Design review of the part built by this model. Coordinates are the model's own, in mm. Face numbers are marked on the shaded views. A direction names the side the tool comes from. Coordinates: 2 decimals unless noted, no trailing zeros. Order: outer loops, then holes, each group sorted by start corner. A loop starts at its lowest first (then second) coordinate and runs counter-clockwise, first axis right, second up. Notation, with made-up numbers: M -1.75,-8.5 L 16.25,-8.5 A3 cw 16.25,-3.5 Z; hole C 8.25,-1.5 d8. An arc over 180 degrees is marked long. Answer as a JSON object with one key per item and string values.
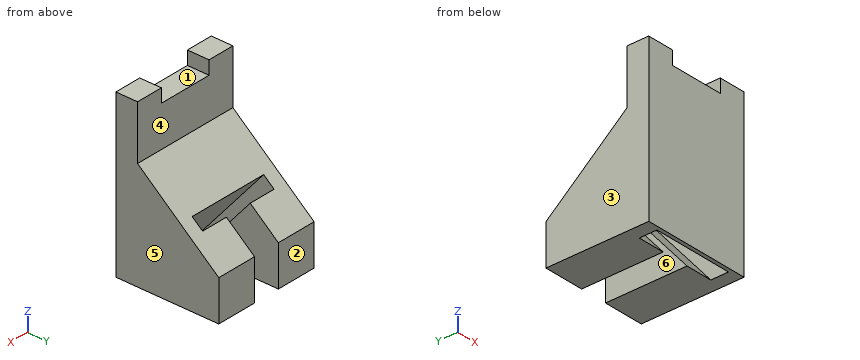
from build123d import *

# Parameters (mm, degrees)
BASE_PLATE_SKETCH_W                   = 40
BASE_PLATE_SKETCH_H                   = 60
BASE_PLATE_60X40X8_DEPTH              = 8
BASE_NOTCH_SKETCH_W                   = 20
BASE_NOTCH_SKETCH_H                   = 5
BASE_NOTCH_20X5_DEPTH                 = 20
UPRIGHT_BLOCK_SKETCH_W                = 40
UPRIGHT_BLOCK_SKETCH_H                = 30
UPRIGHT_BLOCK_40X30X40_DEPTH          = 40
SLOPED_FACE_CUT_DEPTH                 = 40
TOP_SLOT_CUT_DEPTH                    = 39
ANGLED_SLOT_THROUGH_SLOPED_FACE_REACH = 54.383
ANGLED_SLOT_SKETCH_W                  = 10
ANGLED_SLOT_SKETCH_H                  = 15


with BuildPart() as part:
    # Base Plate Sketch → Base Plate 60x40x8 (new body)
    with BuildSketch(Plane(origin=(0, 0, 0), x_dir=(1, 0, 0), z_dir=(0, 1, 0))):
        Rectangle(BASE_PLATE_SKETCH_W, BASE_PLATE_SKETCH_H)
    extrude(amount=BASE_PLATE_60X40X8_DEPTH)

    # Base Notch Sketch → Base Notch 20x5 (cut)
    with BuildSketch(Plane(origin=(0, 8, 0), x_dir=(1, 0, 0), z_dir=(0, 1, 0))):
        with Locations((0, -27.5)):
            Rectangle(BASE_NOTCH_SKETCH_W, BASE_NOTCH_SKETCH_H)
    extrude(amount=-BASE_NOTCH_20X5_DEPTH, mode=Mode.SUBTRACT)

    # Upright Block Sketch → Upright Block 40x30x40 (add)
    with BuildSketch(Plane(origin=(20, 0, 0), x_dir=(0, 0, -1), z_dir=(1, 0, 0))):
        with Locations((10, 23)):
            Rectangle(UPRIGHT_BLOCK_SKETCH_W, UPRIGHT_BLOCK_SKETCH_H)
    extrude(amount=-UPRIGHT_BLOCK_40X30X40_DEPTH)

    # Slope Cut Sketch → Sloped Face Cut (cut)
    with BuildSketch(Plane(origin=(20, 0, 0), x_dir=(0, 0, -1), z_dir=(1, 0, 0))):
        Polygon((15, 38), (-10, 38), (-10, 8), align=None)
    extrude(amount=-SLOPED_FACE_CUT_DEPTH, mode=Mode.SUBTRACT)

    # Top Slot Sketch → Top Slot Cut (cut)
    with BuildSketch(Plane(origin=(0, 8.196721311, 9.836065574), x_dir=(1, 0, 0), z_dir=(0, 0.6401843996644799, 0.768221279597376))):
        Polygon((-5, 25.272676797), (-15, 25.272676797), (-15, 20.272676797), (15, 20.272676797), (15, 25.272676797), (5, 25.272676797), (5, 38.79517462), (-5, 38.79517462), align=None)
    extrude(amount=-TOP_SLOT_CUT_DEPTH, mode=Mode.SUBTRACT)

    # Angled Slot Sketch → Angled Slot Through Sloped Face (cut, up to next)
    with BuildSketch(Plane(origin=(0, 38, 0), x_dir=(1, 0, 0), z_dir=(0, 1, 0)), mode=Mode.PRIVATE) as angled_slot_through_sloped_face_sk1:
        with Locations((0, 22.5)):
            Rectangle(ANGLED_SLOT_SKETCH_W, ANGLED_SLOT_SKETCH_H)
    angled_slot_through_sloped_face_tool1 = extrude(angled_slot_through_sloped_face_sk1.sketch, amount=-ANGLED_SLOT_THROUGH_SLOPED_FACE_REACH, mode=Mode.PRIVATE) & part.part
    add(angled_slot_through_sloped_face_tool1.solids().sort_by_distance((0, 38, -22.5))[0], mode=Mode.SUBTRACT)


solid = part.part
1) Insertion check: pin 1 Ø6 at (x, z) = (-7, 6.5) entering from +Y; pin 2 Ø2.5 at (x, y) = (3, 3) entering from +Z; pin 3 Ø16 at (x, z) = (6, 20.5) entering from +Y. Each pin has a flat end and moves straight along its axis. Give the tip position at first contact, or say it passes through.
Taken from the geometry:
{"pin 1": "stops at y = 15.8", "pin 2": "stops at z = 25", "pin 3": "stops at y = 8"}
2) To check wall thickness, follow L1, parallel to X at y = 29.5, z = -25; L2, parallel to X at y = 10, z = -22; L3, parallel to Y at x = -15.5, z = 18. State the ranges of each line that lie inside material, in increasing order.
Taken from the geometry:
{"L1": "x = -20 to -5, 5 to 20", "L2": "x = -20 to -15, 15 to 20", "L3": "y = 0 to 8"}
3) Mouldability with a two-part tool opening along X and no side actions: class the marked faces 1, 2 and 3 as released by +X, released by -X, zero draft, split by the parting line, or undercut.
Taken from the geometry:
{"face 1": "undercut", "face 2": "zero draft", "face 3": "released by -X"}
4) Add section A-A (x = 13). State the section outline as (y, z) points.
Taken from the geometry:
{"outline": "M 0,-30 L 1.39,-30 L 23.77,-3.14 L 8,10 L 8,30 L 0,30 Z; M 7.9,-30 L 38,-30 L 38,-15 L 27.61,-6.34 Z"}
5) Add section C-C (z = -9.5). State the section outline as (x, y) points.
Taken from the geometry:
{"outline": "M -20,0 L 20,0 L 20,31.4 L 5,31.4 L 5,24.98 L 15,24.98 L 15,18.47 L -15,18.47 L -15,24.98 L -5,24.98 L -5,31.4 L -20,31.4 Z"}
6) Tool access review of the marked faces 4, 5 and 6: name each direction out of +Z, -Z, +X, -X, +Y, -Y from which nothing blocks a thin tool from reaching the whole face with its end or side.
Taken from the geometry:
{"face 4": "+Z, +X, -X, +Y", "face 5": "+Z, -Z, +X, +Y, -Y", "face 6": "-Z, +Y"}
7) Add section D-D (x = 1.5). State the section outline as (y, z) points, and give its area (3 significant figures).
Taken from the geometry:
{"outline": "M 0,-30 L 1.39,-30 L 23.77,-3.14 L 8,10 L 8,25 L 0,25 Z", "area": "667 mm2"}
8) Add section B-B (y = 29). State the section outline as (x, z) points, and give its area (3 significant figures).
Taken from the geometry:
{"outline": "M -20,-30 L -5,-30 L -5,-7.5 L -20,-7.5 Z; M 5,-30 L 20,-30 L 20,-7.5 L 5,-7.5 Z", "area": "675 mm2"}
